Model file for the job. Use its own axes, mm. A direction names the side the tool comes from. Round coordinates to 2 decimals unless told otherwise and drop trailing zeros. Loops run counter-clockwise (first coordinate to the right, second up) from the corner with the lowest first, then second, coordinate; pieces in that order, holes last. Notation, with made-up numbers: (77.5, 74.25) - (122.5, 74.25) arc R29 ccw to (122.5, 107.25) - close; hole circle Ø3 at (43, -31). An arc over 180 degrees is marked (long way). Use one line per item in the form item = value.
from build123d import *

# Parameters (mm, degrees)
BOSS_EXTRUDE1_DEPTH                          = 50
CBORE_FOR_M5_SLOTTED_CHEESE_HEAD_SCR_2_COUNT = 2
CBORE_FOR_M5_SLOTTED_CHEESE_HEAD_SCR_2_PITCH = 35
SKETCH6_W                                    = 45
SKETCH6_H                                    = 25
CUT_EXTRUDE1_DEPTH                           = 1
CHAMFER1_SIZE                                = 0.5


with BuildPart() as part:
    # Sketch2 → Boss-Extrude1 (new body)
    with BuildSketch(Plane.XY):
        Polygon((55, 8), (65, 8), (65, 0), (0, 0), (0, 8), (10, 8), (10, 18), (55, 18), align=None)
    extrude(amount=BOSS_EXTRUDE1_DEPTH)

    # Sketch4 → CBORE for M5 Slotted cheese head screws1 (revolve, cut)
    with BuildSketch(Plane(origin=(15, 0, 37.5), x_dir=(0, 0, -1), z_dir=(1, 0, 0))):
        Polygon((0, 0), (0, 18), (2.75, 18), (2.75, 6), (5, 6), (5, 0.025), (5.025, 0), align=None)
    cbore_for_m5_slotted_cheese_head_screws1 = revolve(axis=Axis((15, -6.35, 37.5), (0, 1, 0)), mode=Mode.SUBTRACT)

    # CBORE for M5 Slotted cheese head scr 2: CBORE for M5 Slotted cheese head screws1 ×2
    with Locations(*[(i * CBORE_FOR_M5_SLOTTED_CHEESE_HEAD_SCR_2_PITCH, 0, 0) for i in range(1, CBORE_FOR_M5_SLOTTED_CHEESE_HEAD_SCR_2_COUNT)]):
        add(cbore_for_m5_slotted_cheese_head_screws1, mode=Mode.SUBTRACT)

    # Sketch6 → Cut-Extrude1 (cut)
    with BuildSketch(Plane(origin=(0, 18, 0), x_dir=(1, 0, 0), z_dir=(0, 1, 0))):
        with Locations((32.5, -37.5)):
            Rectangle(SKETCH6_W, SKETCH6_H)
    extrude(amount=-CUT_EXTRUDE1_DEPTH, mode=Mode.SUBTRACT)

    # Chamfer1
    chamfer1_edges = [part.edges().sort_by_distance(p)[0] for p in [
        (60, 8, 0),
        (65, 4, 0),
        (32.5, 0, 0),
        (0, 4, 0),
        (65, 4, 50),
        (0, 8, 25),
        (65, 8, 25),
        (65, 0, 25),
        (0, 0, 25),
        (60, 8, 50),
        (55, 12.5, 50),
        (5, 8, 50),
        (10, 12.5, 50),
        (10, 18, 12.5),
        (55, 18, 12.5),
        (0, 4, 50),
        (10, 17, 37.5),
        (10, 17.5, 25),
        (55, 17, 37.5),
        (55, 17.5, 25),
        (32.5, 17, 50),
        (5, 8, 0),
        (32.5, 0, 50),
        (10, 13, 0),
        (32.5, 18, 0),
        (55, 13, 0),
    ]]
    chamfer(chamfer1_edges, length=CHAMFER1_SIZE)


solid = part.part
1. Cut at D-D, the plane x = 26. Give the cut face in (y, z).
Geometry check:
outline = (0, 0.5) - (0.5, 0) - (17.5, 0) - (18, 0.5) - (18, 25) - (17, 25) - (17, 49.5) - (16.5, 50) - (0.5, 50) - (0, 49.5) - close
2. Cut at B-B, the plane x = 50. Give the cut face in (y, z) (3 decimals), plus the area to 3 significant figures.
Geometry check:
outline = (0, 0.5) - (0.5, 0) - (17.5, 0) - (18, 0.5) - (18, 25) - (17, 25) - (17, 34.75) - (6, 34.75) - (6, 32.5) - (0.025, 32.5) - (0, 32.475) - close; (0, 42.525) - (0.025, 42.5) - (6, 42.5) - (6, 40.25) - (17, 40.25) - (17, 49.5) - (16.5, 50) - (0.5, 50) - (0, 49.5) - close
area = 754 mm^2
3. Cut at C-C, the plane z = 4. Give the cut face in (x, y), plus the area to 3 significant figures.
Geometry check:
outline = (0, 0.5) - (0.5, 0) - (64.5, 0) - (65, 0.5) - (65, 7.5) - (64.5, 8) - (55, 8) - (55, 17.5) - (54.5, 18) - (10.5, 18) - (10, 17.5) - (10, 8) - (0.5, 8) - (0, 7.5) - close
area = 969 mm^2
4. Cut at A-A, the plane z = 37.5. Give the number of separate pieces and of enclosed holes in the cut face, plus the area to 3 significant figures.
Geometry check:
separate_pieces = 3
enclosed_holes = 0
area = 683 mm^2
5. Flat gauge pins, fed straight in: pin 1 (9 mm diameter, centred on x = 50, z = 37.5, fed in from -Y); pin 2 (7.5 mm diameter, centred on x = 40.5, z = 31.5, fed in from +Y); pin 3 (3 mm diameter, centred on y = 12.5, z = 37, fed in from +X). Where does each tip first touch, or does it go through?
Geometry check:
pin_1 = 6
pin_2 = 17
pin_3 = 55
6. Tool access for faces 1 (the flat face through (32, 17, 37)), 2 (the flat face through (55, 13, 25)), 3 (the cylindrical face through (14.78, 2.971, 42.495)): list every direction of +Z, -Z, +X, -X, +Y, -Y with a clear straight run to the whole face (end or side of a thin tool).
Geometry check:
face_1 = +Z, +X, -X, +Y
face_2 = +Z, -Z, +X, +Y
face_3 = -Y
7. Wall check: probe 1 along X at (y, z) = (2.6, 37.5); probe 2 along Z at (x, y) = (15, 2.55); probe 3 along Z at (x, y) = (50, 14). Give the ranges that are in metal, low to high.
Geometry check:
probe_1 = 0 to 10, 20 to 45, 55 to 65
probe_2 = 0 to 32.5, 42.5 to 50
probe_3 = 0 to 34.75, 40.25 to 50
8. Pull direction X, two halves, no side cores. Call faces 4 (the flat face through (10, 13, 25)), 5 (the flat face through (17, 6, 40)), 6 (the flat face through (65, 4, 25)), 7 (the flat face through (60, 8, 25)): +X half, -X half, draft (parallel to the pull), parting line (faces both ways), or undercut.
Geometry check:
face_4 = -X half
face_5 = undercut
face_6 = +X half
face_7 = draft
